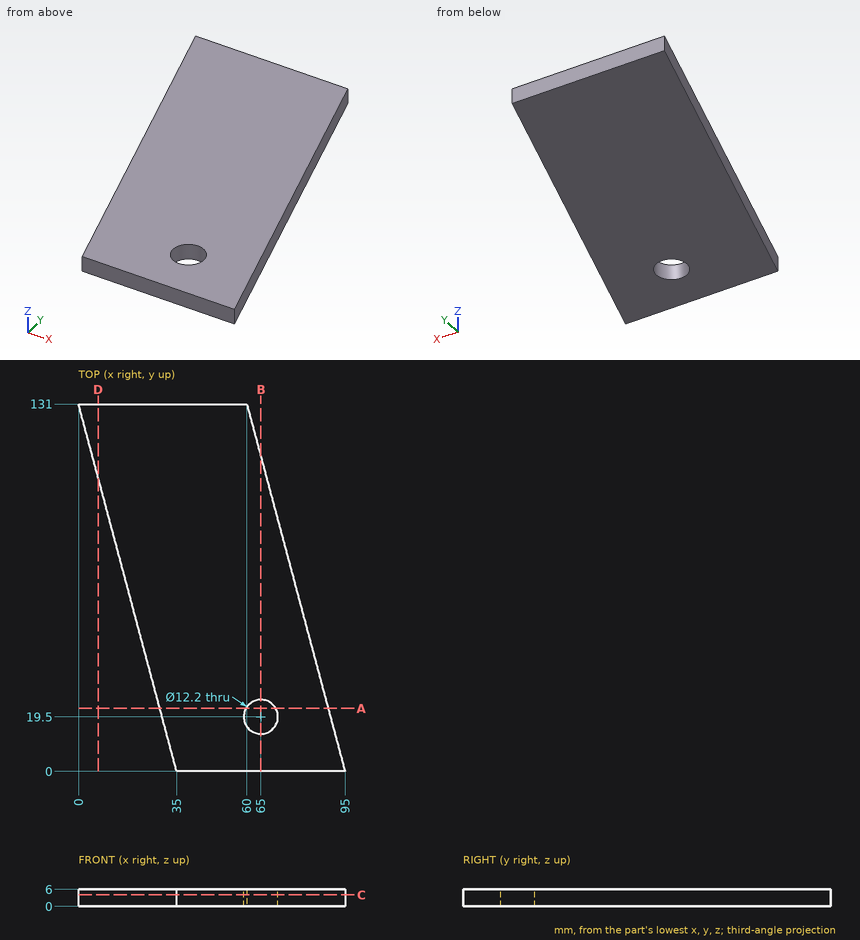
Verification items for this drawing (mm, ordinates from the low corner). Coordinates: 2 decimals unless noted, no trailing zeros. Loops run counter-clockwise (first coordinate to the right, second up) from the corner with the lowest first, then second, coordinate; pieces in that order, holes last. Notation, with made-up numbers: (20, -28.75) -> (68, -28.75) arc R21 cw to (68, -14.75) -> close; hole circle Ø5 at (84, 41). An arc over 180 degrees is marked (long way). Answer in a Markdown table with one row per item. Add a question column.
1. Section check B-B, the plane x = 65. Enter the section's corners in (y, z).
2. Section check C-C, the plane z = 4.05. Enter the section's corners in (x, y).
3. Section check A-A, the plane y = 22.5. Enter the section's corners in (x, z).
4. Material ranges on probe 1 along X at (y, z) = (19.5, 2.65); probe 2 along X at (y, z) = (50, 3.5); probe 3 along X at (y, z) = (106.5, 1.7), recorded low to high. Write a range as [from, to].
5. Section check D-D, the plane x = 7. Enter the section's corners in (y, z).
6. Depth check by flat-ended pin: P1, Ø1.5, axis at y = 35.5, z = 3, coming from the +X side; P2, Ø2, axis at y = 66, z = 4, coming from the +X side; P3, Ø3, axis at y = 59, z = 2, coming from the -X side. Enter the tip coordinate at first touch or a pass-through.
Derived:
| question | item | result |
|---|---|---|
| 1 | outline | (0, 0) -> (13.4, 0) -> (13.4, 6) -> (0, 6) -> close; (25.6, 0) -> (112.29, 0) -> (112.29, 6) -> (25.6, 6) -> close |
| 2 | outline | (0, 131) -> (35, 0) -> (95, 0) -> (60, 131) -> close; hole circle Ø12.2 at (65, 19.5) |
| 3 | outline | (28.99, 0) -> (59.69, 0) -> (59.69, 6) -> (28.99, 6) -> close; (70.31, 0) -> (88.99, 0) -> (88.99, 6) -> (70.31, 6) -> close |
| 4 | probe 1 | x = [29.79, 58.9], [71.1, 89.79] |
| 4 | probe 2 | x = [21.64, 81.64] |
| 4 | probe 3 | x = [6.55, 66.55] |
| 5 | outline | (104.8, 0) -> (131, 0) -> (131, 6) -> (104.8, 6) -> close |
| 6 | P1 | stops at x = 85.72 |
| 6 | P2 | stops at x = 77.63 |
| 6 | P3 | stops at x = 18.84 |
